Check sheet for the modelled part. Datum: model origin and axes. Units: mm. Coordinates: 2 decimals unless noted, no trailing zeros. Loops run counter-clockwise (first coordinate to the right, second up) from the corner with the lowest first, then second, coordinate; pieces in that order, holes last. Notation, with made-up numbers: (20.5, 60.5) - (30.5, 60.5) arc R35 ccw to (30.5, 98.5) - close; hole circle Ø9 at (-22, -18.5). An arc over 180 degrees is marked (long way). Use a Markdown table: item, result. Add a question column.
1) Sectioned sample at C-C, the plane x = 18.5. Enter the section's corners in (y, z).
2) Thickness scan on line 1 (Y direction, x = 20, z = 5.75); line 2 (X direction, y = 30, z = 4.5); line 3 (Y direction, x = 26.5, z = 1.25). Record the ranges inside material, lowest first.
3) Sectioned sample at B-B, the plane x = 85.5. Enter the section's corners in (y, z).
4) Sectioned sample at A-A, the plane z = 7. Enter the section's corners in (x, y).
5) Go/stop test with a flat-tipped pin: P1, Ø12, axis at x = 23.5, y = 74.5, coming from the -Z side. Record where the tip stops, or that it passes through.
from build123d import *

# Parameters (mm, degrees)
SKETCH_1_W          = 100
SKETCH_1_H          = 120
EXTRUDE_1_DEPTH     = 10
CUT_EXTRUDE_1_DEPTH = 10
SKETCH_3_W          = 100
SKETCH_3_H          = 120
CUT_EXTRUDE_2_DEPTH = 10


with BuildPart() as part:
    # Sketch 1 → Extrude 1 (new body)
    with BuildSketch(Plane.XY):
        with Locations((50, 60)):
            Rectangle(SKETCH_1_W, SKETCH_1_H)
    extrude(amount=EXTRUDE_1_DEPTH)

    # Sketch 2 → Cut-Extrude 1 (cut)
    with BuildSketch(Plane.XY.offset(10)):
        with BuildLine():
            ThreePointArc((87.5, 90), (80, 97.5), (72.5, 90))
            Line((72.5, 90), (80, 90))
            Line((80, 90), (80, 82.5))
            ThreePointArc((80, 82.5), (85.303300859, 84.696699141), (87.5, 90))
        make_face()
        with BuildLine():
            Line((80, 90), (72.5, 90))
            ThreePointArc((72.5, 90), (74.696699141, 84.696699141), (80, 82.5))
            Line((80, 82.5), (80, 90))
        make_face()
        with BuildLine():
            ThreePointArc((27.5, 90), (14.696699141, 95.303300859), (20, 82.5))
            Line((20, 82.5), (20, 90))
            Line((20, 90), (27.5, 90))
        make_face()
        with BuildLine():
            Line((20, 90), (20, 82.5))
            ThreePointArc((20, 82.5), (25.303300859, 84.696699141), (27.5, 90))
            Line((27.5, 90), (20, 90))
        make_face()
        with BuildLine():
            ThreePointArc((27.5, 30), (25.303300859, 35.303300859), (20, 37.5))
            Line((20, 37.5), (20, 30))
            Line((20, 30), (27.5, 30))
        make_face()
        with BuildLine():
            Line((20, 30), (20, 37.5))
            ThreePointArc((20, 37.5), (14.696699141, 24.696699141), (27.5, 30))
            Line((27.5, 30), (20, 30))
        make_face()
        with BuildLine():
            ThreePointArc((80, 37.5), (74.696699141, 35.303300859), (72.5, 30))
            Line((72.5, 30), (80, 30))
            Line((80, 30), (80, 37.5))
        make_face()
        with BuildLine():
            Line((80, 30), (72.5, 30))
            ThreePointArc((72.5, 30), (80, 22.5), (87.5, 30))
            ThreePointArc((87.5, 30), (85.303300859, 35.303300859), (80, 37.5))
            Line((80, 37.5), (80, 30))
        make_face()
    extrude(amount=-CUT_EXTRUDE_1_DEPTH, mode=Mode.SUBTRACT)

    # Sketch 3 → Cut-Extrude 2 (cut)
    with BuildSketch(Plane.XY.offset(10)):
        with Locations((50, 60)):
            Rectangle(SKETCH_3_W, SKETCH_3_H)
        Polygon((95, 60), (95, 5), (5, 5), (5, 115), (95, 115), align=None, mode=Mode.SUBTRACT)
    extrude(amount=-CUT_EXTRUDE_2_DEPTH, mode=Mode.SUBTRACT)


solid = part.part
Solved:
| question | item | result |
|---|---|---|
| 1 | outline | (5, 0) - (22.65, 0) - (22.65, 10) - (5, 10) - close; (37.35, 0) - (82.65, 0) - (82.65, 10) - (37.35, 10) - close; (97.35, 0) - (115, 0) - (115, 10) - (97.35, 10) - close |
| 2 | line 1 | y = 5 to 22.5, 37.5 to 82.5, 97.5 to 115 |
| 2 | line 2 | x = 5 to 12.5, 27.5 to 72.5, 87.5 to 95 |
| 2 | line 3 | y = 5 to 26.26, 33.74 to 86.26, 93.74 to 115 |
| 3 | outline | (5, 0) - (24.9, 0) - (24.9, 10) - (5, 10) - close; (35.1, 0) - (84.9, 0) - (84.9, 10) - (35.1, 10) - close; (95.1, 0) - (115, 0) - (115, 10) - (95.1, 10) - close |
| 4 | outline | (5, 5) - (95, 5) - (95, 115) - (5, 115) - close; hole circle Ø15 at (20, 30); hole circle Ø15 at (20, 90); hole circle Ø15 at (80, 30); hole circle Ø15 at (80, 90) |
| 5 | P1 | stops at z = 0 |
